from build123d import *

# Parameters (mm, degrees)
SKETCH_1_W               = 90
SKETCH_1_H               = 90
EXTRUDE_1_DEPTH          = 8
SKETCH_2_R               = 45
EXTRUDE_2_DEPTH          = 100
SKETCH_3_W               = 90
SKETCH_3_H               = 90
EXTRUDE_3_DEPTH          = 29
SKETCH_4_R               = 6
EXTRUDE_4_DEPTH          = 37
SKETCH_6_W               = 75
SKETCH_6_H               = 49
EXTRUDE_5_DEPTH          = 80
SKETCH_7_R               = 3.5
CUT_EXTRUDE_1_DEPTH      = 8
FILLET_1_R               = 5
FILLET_2_R               = 5
SKETCH_9_W               = 30
SKETCH_9_H               = 15.937749453
CUT_EXTRUDE_2_DEPTH      = 1
PATTERN_CIRCULAR_1_COUNT = 4


with BuildPart() as part:
    # 草图1 → 凸台-拉伸1 (new body)
    with BuildSketch(Plane.XY):
        Rectangle(SKETCH_1_W, SKETCH_1_H)
    extrude(amount=EXTRUDE_1_DEPTH)

    # 草图2 → 凸台-拉伸2 (add)
    with BuildSketch(Plane(origin=(0, 0, 0), x_dir=(-1, 0, 0), z_dir=(0, 0, -1))):
        Circle(SKETCH_2_R)
    extrude(amount=EXTRUDE_2_DEPTH)

    # 草图3 → 凸台-拉伸3 (add)
    with BuildSketch(Plane(origin=(0, 0, -100), x_dir=(-1, 0, 0), z_dir=(0, 0, -1))):
        Rectangle(SKETCH_3_W, SKETCH_3_H)
    extrude(amount=EXTRUDE_3_DEPTH)

    # 草图4 → 凸台-拉伸4 (add)
    with BuildSketch(Plane.XY.offset(8)):
        Circle(SKETCH_4_R)
    extrude(amount=EXTRUDE_4_DEPTH)

    # 草图6 → 凸台-拉伸5 (add)
    with BuildSketch(Plane(origin=(0, 0, 0), x_dir=(0, 0, -1), z_dir=(1, 0, 0))):
        with Locations((34.5, 0)):
            Rectangle(SKETCH_6_W, SKETCH_6_H)
    extrude(amount=EXTRUDE_5_DEPTH)

    # 草图7 → 切除-拉伸1 (cut)
    with BuildSketch(Plane.XY.offset(8)):
        with Locations((-36.769552622, 36.769552622)):
            Circle(SKETCH_7_R)
    cut_extrude_1 = extrude(amount=-CUT_EXTRUDE_1_DEPTH, mode=Mode.SUBTRACT)

    # 圆角1
    fillet_1_edges = [part.edges().sort_by_distance(p)[0] for p in [
        (-45, 45, 4),
        (45, 45, 4),
        (45, -45, 4),
        (-45, -45, 4),
    ]]
    fillet(fillet_1_edges, radius=FILLET_1_R)

    # 圆角2
    fillet_2_edges = [part.edges().sort_by_distance(p)[0] for p in [
        (45, 45, -114.5),
        (45, -45, -114.5),
        (-45, -45, -114.5),
        (-45, 45, -114.5),
    ]]
    fillet(fillet_2_edges, radius=FILLET_2_R)

    # 草图9 → 切除-拉伸2 (cut)
    with BuildSketch(Plane(origin=(6, 0, 0), x_dir=(0, 0, -1), z_dir=(1, 0, 0))):
        with Locations((-30, -0.084649365)):
            Rectangle(SKETCH_9_W, SKETCH_9_H)
    extrude(amount=-CUT_EXTRUDE_2_DEPTH, mode=Mode.SUBTRACT)

    # 阵列(圆周)1: 切除-拉伸1 ×4 about axis
    pattern_circular_1_axis = Axis((0, 0, 0), (0, 0, 1))
    for i in range(1, PATTERN_CIRCULAR_1_COUNT):
        add(cut_extrude_1.rotate(pattern_circular_1_axis, i * 360 / PATTERN_CIRCULAR_1_COUNT), mode=Mode.SUBTRACT)


solid = part.part
Work out the finished part from the listing and answer in its coordinate system (mm). A direction names the side the tool comes from. Give positions to 0.01 mm unless a question says otherwise; leave off trailing zeros. Write each loop counter-clockwise with the first axis right and the second up, starting at its lowest first coordinate (ties: lowest second). Pieces come first, ordered by that corner, then holes. Notation, with made-up numbers: (37.5, -5) - (77.5, -5) arc R22 cw to (77.5, 21) - close; hole circle Ø8 at (35, 57). An arc over 180 degrees is marked (long way). One line per item, written item: value. Start each with the question number.
1. Given pin 1 (2 mm diameter, centred on y = 1, z = 26, fed in from +X); pin 2 (0.8 mm diameter, centred on x = 5.5, y = 0.5, fed in from +Z); pin 3 (2.5 mm diameter, centred on y = 6.5, z = 5.5, fed in from +X), each flat-ended and moving along its own axis, determine where each tip first touches the part or whether it passes through.
2. For a pull along Z with two mould halves and no side action, classify faces 6 (the flat face through (-1, 11, 8)), 7 (the flat face through (-34, -36, -100)), 8 (the flat face through (45, -1, -114)) as +Z half, -Z half, draft (parallel to the pull), parting line (faces both ways), or undercut.
3. Find section A-A (z = -102.5). Write down the section's boundary in (x, y).
4. Consider probe 1 along Z at (x, y) = (-39, 28); probe 2 along X at (y, z) = (-23, -119); probe 3 along Z at (x, y) = (-36, 24.5). Determine where each line is inside the solid, lowest interval first.
5. For faces 1 (the flat face through (34, -34, -100)), 2 (the flat face through (-34, 36, -100)), 3 (the flat face through (5, 0, 30)), 4 (the cylindrical face through (39.135, 39.349, 4.056)), 5 (the flat face through (32, 37, 0)), determine the directions among +Z, -Z, +X, -X, +Y, -Y from which every point of the face is accessible in a straight line to the end or side of a thin tool.
6. Find section B-B (x = 27). Write down the section's boundary in (y, z), then the cut area to 3 significant figures.
7. Find section C-C (y = -12). Write down the section's boundary in (x, z), then the cut area to 3 significant figures.
8. Find section D-D (z = -40.5). Write down the section's boundary in (x, y), then the cut area to 3 significant figures.
Geometry results:
1. pin 1: x = 5
1. pin 2: z = 15
1. pin 3: x = 45
2. face 6: +Z half
2. face 7: undercut
2. face 8: draft
3. outline: (-45, -40) arc R5 ccw to (-40, -45) - (40, -45) arc R5 ccw to (45, -40) - (45, 40) arc R5 ccw to (40, 45) - (-40, 45) arc R5 ccw to (-45, 40) - close
4. probe 1: -129 to -100, 0 to 8
4. probe 2: -45 to 45
4. probe 3: -129 to 8
5. face 1: +X, -Y
5. face 2: -X, +Y
5. face 3: +Z, +X, +Y, -Y
5. face 4: +Z
5. face 5: +X, +Y
6. outline: (-45, -129) - (45, -129) - (45, -100) - (36, -100) - (36, 0) - (45, 0) - (45, 8) - (-45, 8) - (-45, 0) - (-36, 0) - (-36, -100) - (-45, -100) - close
6. area: 10,500 mm2
7. outline: (-45, -129) - (45, -129) - (45, -100) - (43.37, -100) - (43.37, -72) - (80, -72) - (80, 3) - (45, 3) - (45, 8) - (-45, 8) - (-45, 0) - (-43.37, 0) - (-43.37, -100) - (-45, -100) - close
7. area: 14,700 mm2
8. outline: (37.75, -24.5) - (80, -24.5) - (80, 24.5) - (37.75, 24.5) arc R45 ccw (long way) to start
8. area: 8,190 mm2
